The model under review builds one solid part; all positions refer to its coordinate system, in mm. Coordinates: 2 decimals unless noted, no trailing zeros. Loops run counter-clockwise (first coordinate to the right, second up) from the corner with the lowest first, then second, coordinate; pieces in that order, holes last. Notation, with made-up numbers: (2.25, 88.25) - (7.25, 88.25) arc R25 ccw to (7.25, 102.25) - close; hole circle Ø1 at (-25.5, 62.5). An arc over 180 degrees is marked (long way). Answer in a Markdown table with one row per item. Add a question column.
(1) For line 1 along Y through (x, z) = (0, -10); line 2 along Y through (x, z) = (-6.75, 16.5), list the stretches that pass through material, from the lowest coordinate up.
(2) We need section A-A on x = 0. Write out the cut boundary in (y, z), plus the area to 3 significant figures.
(3) We need section C-C on z = 21. Write out the cut boundary in (x, y), plus the area to 3 significant figures.
(4) Mouldability with a two-part tool opening along X and no side actions: class faces 1 (the cylindrical face through (-9.468, 3.926, -0.35)), 2 (the cylindrical face through (-8.06, -12.65, 0.35)), 3 (the flat face through (0.1, -11.5, -26)) as +X half, -X half, draft (parallel to the pull), parting line (faces both ways), or undercut.
(5) For P1, Ø4, axis at x = -5.5, z = -18.5, coming from the -Y side; P2, Ø12, axis at y = 9.5, z = 12, coming from the +X side; P3, Ø1, axis at y = -3, z = -6, coming from the +X side, all flat-tipped, find the tip position at first contact; note any pin that passes through.
from build123d import *

# Parameters (mm, degrees)
SKETCH_1_R      = 15
SKETCH_1_R_2    = 10.25
EXTRUDE_1_DEPTH = 26
CHAMFER_1_SIZE  = 1


with BuildPart() as part:
    # 草图1 → 凸台-拉伸1 (new, symmetric)
    with BuildSketch(Plane.XY):
        with Locations(Location((0, 0, 0), (0, 0, 180))):
            Circle(SKETCH_1_R)
        with Locations(Location((0, 0, 0), (0, 0, 180))):
            Circle(SKETCH_1_R_2, mode=Mode.SUBTRACT)
    extrude(amount=EXTRUDE_1_DEPTH, both=True)

    # 倒角1
    chamfer_1_edges = [part.edges().sort_by_distance(p)[0] for p in [
        (15, 0, -26),
        (15, 0, 26),
        (10.25, 0, -26),
        (10.25, 0, 26),
    ]]
    chamfer(chamfer_1_edges, length=CHAMFER_1_SIZE)


solid = part.part
Outcome:
| question | item | result |
|---|---|---|
| 1 | line 1 | -15 to -10.25, 10.25 to 15 |
| 1 | line 2 | -13.4 to -7.71, 7.71 to 13.4 |
| 2 | outline | (-15, -25) - (-14, -26) - (-11.25, -26) - (-10.25, -25) - (-10.25, 25) - (-11.25, 26) - (-14, 26) - (-15, 25) - close; (10.25, -25) - (11.25, -26) - (14, -26) - (15, -25) - (15, 25) - (14, 26) - (11.25, 26) - (10.25, 25) - close |
| 2 | area | 490 mm² |
| 3 | outline | circle Ø30 at (0, 0); hole circle Ø20.5 at (0, 0) |
| 3 | area | 377 mm² |
| 4 | face 1 | undercut |
| 4 | face 2 | parting line |
| 4 | face 3 | draft |
| 5 | P1 | y = -14.59 |
| 5 | P2 | x = 14.59 |
| 5 | P3 | x = 14.79 |
